from build123d import *

# Parameters (mm, degrees)
HOLE_WIZARD_M4_1_D  = 3.3
CUT_EXTRUDE_1_DEPTH = 10
FILLET_1_R          = 10
CUT_EXTRUDE_2_DEPTH = 10
CHAMFER_1_SIZE      = 0.2


with BuildPart() as part:
    # 草图1 → 旋转1 (revolve)
    with BuildSketch(Plane(origin=(0, 0, 0), x_dir=(1, 0, 0), z_dir=(0, 1, 0)), mode=Mode.PRIVATE) as revolve_1_sk:
        Polygon((0, 23.5), (0, 35), (4, 35), (4, 27.5), (8, 27.5), (8, 25.5), (3, 25.5), (3, 23.5), align=None)
    revolve(revolve_1_sk.sketch.rotate(Axis((-554.392054902, 0, 0), (1, 0, 0)), 180), axis=Axis((-554.392054902, 0, 0), (1, 0, 0)))

    # M4 螺纹孔1 (through all)
    with Locations(Plane(origin=(4, 0, 0), x_dir=(0, 0, -1), z_dir=(1, 0, 0))):
        with Locations((0, 0), (0, 31), (26.846787517, 15.5), (26.846787517, -15.5), (0, -31), (-26.846787517, -15.5), (-26.846787517, 15.5)):
            Hole(HOLE_WIZARD_M4_1_D / 2)

    # 草图4 → 切除-拉伸1 (cut)
    with BuildSketch(Plane(origin=(4, 0, 0), x_dir=(0, 0, -1), z_dir=(1, 0, 0))):
        with BuildLine():
            Line((-31, -16.248076809), (-31, 16.248076809))
            ThreePointArc((-31, 16.248076809), (-35, 0), (-31, -16.248076809))
        make_face()
    extrude(amount=-CUT_EXTRUDE_1_DEPTH, mode=Mode.SUBTRACT)

    # 圆角1
    fillet_1_edges = [part.edges().sort_by_distance(p)[0] for p in [
        (2, 16.248076809, 31),
        (2, -16.248076809, 31),
    ]]
    fillet(fillet_1_edges, radius=FILLET_1_R)

    # 草图5 → 切除-拉伸2 (cut)
    with BuildSketch(Plane(origin=(4, 0, 0), x_dir=(0, 0, -1), z_dir=(1, 0, 0))):
        with BuildLine():
            ThreePointArc((23.334523779, 23.334523779), (16.5, 28.578838325), (8.541028488, 31.875552268))
            ThreePointArc((8.541028488, 31.875552268), (6.091538746, 30.461338705), (7.505752308, 28.011848962))
            ThreePointArc((7.505752308, 28.011848962), (14.5, 25.11473671), (20.506096654, 20.506096654))
            ThreePointArc((20.506096654, 20.506096654), (23.334523779, 20.506096654), (23.334523779, 23.334523779))
        make_face()
        with BuildLine():
            ThreePointArc((31.875552268, -8.541028488), (33, 0), (31.875552268, 8.541028488))
            ThreePointArc((31.875552268, 8.541028488), (29.426062525, 9.955242051), (28.011848962, 7.505752308))
            ThreePointArc((28.011848962, 7.505752308), (29, 0), (28.011848962, -7.505752308))
            ThreePointArc((28.011848962, -7.505752308), (29.426062525, -9.955242051), (31.875552268, -8.541028488))
        make_face()
        with BuildLine():
            ThreePointArc((8.541028488, -31.875552268), (16.5, -28.578838325), (23.334523779, -23.334523779))
            ThreePointArc((23.334523779, -23.334523779), (23.334523779, -20.506096654), (20.506096654, -20.506096654))
            ThreePointArc((20.506096654, -20.506096654), (14.5, -25.11473671), (7.505752308, -28.011848962))
            ThreePointArc((7.505752308, -28.011848962), (6.091538746, -30.461338705), (8.541028488, -31.875552268))
        make_face()
        with BuildLine():
            ThreePointArc((-23.334523779, -23.334523779), (-16.5, -28.578838325), (-8.541028488, -31.875552268))
            ThreePointArc((-8.541028488, -31.875552268), (-6.091538746, -30.461338705), (-7.505752308, -28.011848962))
            ThreePointArc((-7.505752308, -28.011848962), (-14.5, -25.11473671), (-20.506096654, -20.506096654))
            ThreePointArc((-20.506096654, -20.506096654), (-23.334523779, -20.506096654), (-23.334523779, -23.334523779))
        make_face()
        with BuildLine():
            ThreePointArc((-8.541028488, 31.875552268), (-16.5, 28.578838325), (-23.334523779, 23.334523779))
            ThreePointArc((-23.334523779, 23.334523779), (-23.334523779, 20.506096654), (-20.506096654, 20.506096654))
            ThreePointArc((-20.506096654, 20.506096654), (-14.5, 25.11473671), (-7.505752308, 28.011848962))
            ThreePointArc((-7.505752308, 28.011848962), (-6.091538746, 30.461338705), (-8.541028488, 31.875552268))
        make_face()
    extrude(amount=-CUT_EXTRUDE_2_DEPTH, mode=Mode.SUBTRACT)

    # 倒角1
    chamfer_1_edges = [part.edges().sort_by_distance(p)[0] for p in [
        (8, 0, -25.5),
    ]]
    chamfer(chamfer_1_edges, length=CHAMFER_1_SIZE)


solid = part.part
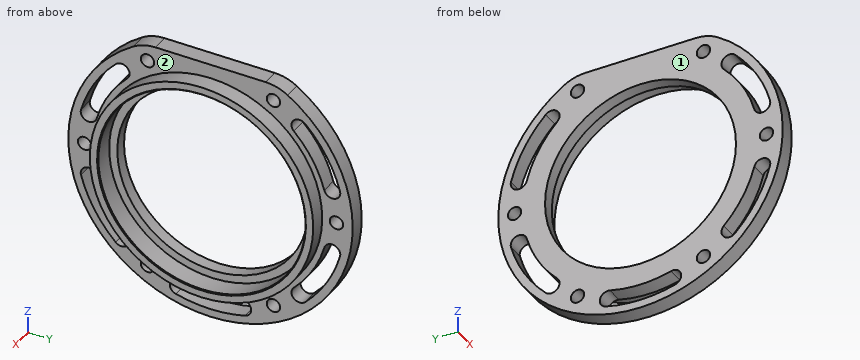
The model under review builds one solid part; all positions refer to its coordinate system, in mm. Face numbers are marked on the shaded views. A direction names the side the tool comes from. Round coordinates to 2 decimals unless told otherwise and drop trailing zeros. Loops run counter-clockwise (first coordinate to the right, second up) from the corner with the lowest first, then second, coordinate; pieces in that order, holes last. Notation, with made-up numbers: (13, -27) -> (69, -27) arc R19 ccw to (69, -5) -> close; hole circle Ø9 at (45, -15). An arc over 180 degrees is marked (long way). One line per question, with ' | ' between items. Start each with the question number.
Item 1: Add section C-C, the plane z = 26.5. Write out the cut boundary in (x, y), then the cut area to 3 significant figures.
Item 2: Add section A-A, the plane y = 0. Write out the cut boundary in (x, z).
Item 3: Machinability: for the marked faces 1 and 2, which of the approach directions +Z, -Z, +X, -X, +Y, -Y give a long, thin tool a straight path to every point of the face, cutting with its end or side? Answer none if there is none.
Item 4: Add section D-D, the plane x = 5.5. Write out the cut boundary in (y, z).
Item 5: Add section B-B, the plane z = 0. Write out the cut boundary in (x, y).
Item 6: Wall thickness on line 1 along Y through (x, z) = (1, 0); line 2 along Z through (x, y) = (1.5, -16.5); line 3 along Z through (x, y) = (1.75, 2): over which ranges is each line inside the solid? List them lowest first. Write a range as [from, to].
Item 7: For pin 1 (1.5 mm diameter, centred on x = 1, z = -14, fed in from -Y) (3 decimals); pin 2 (4 mm diameter, centred on y = -15.5, z = -26.85, fed in from -X); pin 3 (3 mm diameter, centred on x = 5, z = -16, fed in from -Y); pin 4 (5.5 mm diameter, centred on y = 15.5, z = 26.85, fed in from +X), all flat-tipped, find the tip position at first contact; note any pin that passes through.
Return value:
1) outline: (0, -22.86) -> (4, -22.86) -> (4, -17.11) -> (0, -17.11) -> close; (0, -13.89) -> (4, -13.89) -> (4, -7.35) -> (8, -7.35) -> (8, 7.35) -> (4, 7.35) -> (4, 13.89) -> (0, 13.89) -> close; (0, 17.11) -> (4, 17.11) -> (4, 22.86) -> (0, 22.86) -> close | area: 216 mm2
2) outline: (0, -35) -> (4, -35) -> (4, -33) -> (0, -33) -> close; (0, -29) -> (4, -29) -> (4, -27.5) -> (8, -27.5) -> (8, -25.7) -> (7.8, -25.5) -> (3, -25.5) -> (3, -23.5) -> (0, -23.5) -> close; (0, 23.5) -> (3, 23.5) -> (3, 25.5) -> (7.8, 25.5) -> (8, 25.7) -> (8, 27.5) -> (4, 27.5) -> (4, 31) -> (0, 31) -> close
3) face 1: +Z, -Z, -X, +Y, -Y | face 2: +X
4) outline: circle Ø55 at (0, 0); hole circle Ø51 at (0, 0)
5) outline: (0, -35) -> (4, -35) -> (4, -32.65) -> (0, -32.65) -> close; (0, -29.35) -> (4, -29.35) -> (4, -27.5) -> (8, -27.5) -> (8, -25.7) -> (7.8, -25.5) -> (3, -25.5) -> (3, -23.5) -> (0, -23.5) -> close; (0, 23.5) -> (3, 23.5) -> (3, 25.5) -> (7.8, 25.5) -> (8, 25.7) -> (8, 27.5) -> (4, 27.5) -> (4, 29.35) -> (0, 29.35) -> close; (0, 32.65) -> (4, 32.65) -> (4, 35) -> (0, 35) -> close
6) line 1: y = [-35, -32.65], [-29.35, -23.5], [23.5, 29.35], [32.65, 35] | line 2: z = [-30.87, -28.16], [-25.53, -16.73], [16.73, 25.53], [28.16, 30.56] | line 3: z = [-34.94, -32.94], [-28.93, -23.41], [23.41, 31]
7) pin 1: stops at y = -32.395 | pin 2: stops at x = 0 | pin 3: stops at y = -31.68 | pin 4: stops at x = 4
